```python
from build123d import *

# Parameters (mm, degrees)
BASE_BLOCK_SKETCH_W    = 40
BASE_BLOCK_SKETCH_H    = 20
BASE_BLOCK_DEPTH       = 14
UPRIGHT_SKETCH_W       = 30
UPRIGHT_SKETCH_H       = 20
UPRIGHT_BLOCK_DEPTH    = 51
ANGLED_CUT_30DEG_DEPTH = 51
UPPER_LUG_SKETCH_R     = 3
UPPER_LUG_DEPTH        = 5
LOWER_LUG_SKETCH_R     = 3.5
LOWER_LUG_DEPTH        = 5


with BuildPart() as part:
    # Base Block Sketch → Base Block (new body)
    with BuildSketch(Plane(origin=(0, 0, 0), x_dir=(1, 0, 0), z_dir=(0, 1, 0))):
        with Locations((20, -10)):
            Rectangle(BASE_BLOCK_SKETCH_W, BASE_BLOCK_SKETCH_H)
    extrude(amount=BASE_BLOCK_DEPTH)

    # Upright Sketch → Upright Block (add)
    with BuildSketch(Plane(origin=(0, 14, 0), x_dir=(1, 0, 0), z_dir=(0, 1, 0))):
        with Locations((25, -10)):
            Rectangle(UPRIGHT_SKETCH_W, UPRIGHT_SKETCH_H)
    extrude(amount=UPRIGHT_BLOCK_DEPTH)

    # Angled Cut Sketch 30deg → Angled Cut 30deg (cut)
    with BuildSketch(Plane.XY.offset(20)):
        Polygon((10, 65), (10, 35), (27.320508076, 65), align=None)
    extrude(amount=-ANGLED_CUT_30DEG_DEPTH, mode=Mode.SUBTRACT)

    # Upper Lug Sketch → Upper Lug (add)
    with BuildSketch(Plane.XY.offset(20)):
        with BuildLine():
            Line((27.320508076, 65), (27.320508076, 29.29250995))
            Line((27.320508076, 29.29250995), (75.278835908, 51.655845491))
            ThreePointArc((75.278835908, 51.655845491), (79.154580126, 59.515077298), (72.320508076, 65))
            Line((72.320508076, 65), (27.320508076, 65))
        make_face()
        with Locations((72.320508076, 58)):
            Circle(UPPER_LUG_SKETCH_R, mode=Mode.SUBTRACT)
    extrude(amount=UPPER_LUG_DEPTH)

    # Lower Lug Sketch → Lower Lug (add)
    with BuildSketch(Plane(origin=(0, 0, 0), x_dir=(-1, 0, 0), z_dir=(0, 0, -1))):
        with BuildLine():
            Line((-10, 14), (-55, 14))
            ThreePointArc((-55, 14), (-62, 7), (-55, 0))
            Line((-55, 0), (-10, 0))
            Line((-10, 0), (-10, 14))
        make_face()
        with Locations((-55, 7)):
            Circle(LOWER_LUG_SKETCH_R, mode=Mode.SUBTRACT)
    extrude(amount=LOWER_LUG_DEPTH)


solid = part.part
```
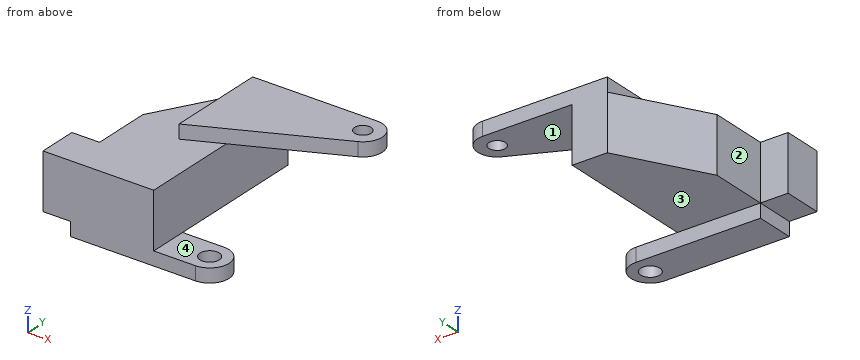
Check sheet for the modelled part. Datum: model origin and axes. Units: mm. Face numbers are marked on the shaded views. A direction names the side the tool comes from. Coordinates: 2 decimals unless noted, no trailing zeros. Write each loop counter-clockwise with the first axis right and the second up, starting at its lowest first coordinate (ties: lowest second). Pieces come first, ordered by that corner, then holes. Notation, with made-up numbers: (-18.5, 68) -> (5.5, 68) arc R29 cw to (5.5, 107) -> close; hole circle Ø10 at (59.5, 69.5). An arc over 180 degrees is marked (long way). Use a Markdown table: item, result.
1. Tool access check on the marked faces 1, 2, 3 and 4. Record the directions out of +Z, -Z, +X, -X, +Y, -Y that give a thin tool (end or side, any length) a straight path to the whole face; none if there is none.
Reported:
| item | result |
|---|---|
| face 1 | -Z, +X, +Y, -Y |
| face 2 | +Z, -Z, -X, +Y |
| face 3 | -Z, +X, -X, +Y |
| face 4 | +Z, +X, +Y, -Y |
2. Go/stop test with flat-tipped pins: pin 1 Ø1 at (y, z) = (44.5, 13) entering from +X; pin 2 Ø4 at (x, z) = (42.5, -1.5) entering from +Y; pin 3 Ø12 at (x, y) = (30, 23.5) entering from +Z; pin 4 Ø9 at (x, y) = (55, 7) entering from -Z. Record where each tip stops, or that it passes through.
Reported:
| item | result |
|---|---|
| pin 1 | stops at x = 40 |
| pin 2 | stops at y = 14 |
| pin 3 | stops at z = 20 |
| pin 4 | stops at z = -5 |
3. Sectioned sample at A-A (y = 7). Enter the section's corners in (x, z), plus the area to 4 significant figures.
Reported:
| item | result |
|---|---|
| outline | (0, 0) -> (10, 0) -> (10, -5) -> (51.5, -5) -> (51.5, 0) -> (40, 0) -> (40, 20) -> (0, 20) -> close; (58.5, -5) -> (62, -5) -> (62, 0) -> (58.5, 0) -> close |
| area | 1,025 mm2 |
4. Sectioned sample at B-B (z = -2). Enter the section's corners in (x, y), plus the area to 3 significant figures.
Reported:
| item | result |
|---|---|
| outline | (10, 0) -> (55, 0) arc R7 ccw to (55, 14) -> (10, 14) -> close; hole circle Ø7 at (55, 7) |
| area | 668 mm2 |
5. Scan lines: line 1 along Y through (x, z) = (55, -2.1); line 2 along Z through (x, y) = (65, 47); line 3 along X through (y, z) = (30.5, 2.75). Record each from-to range of solid material in increasing order.
Reported:
| item | result |
|---|---|
| line 1 | y = 0 to 3.5, 10.5 to 14 |
| line 2 | z = 20 to 25 |
| line 3 | x = 10 to 40 |
6. Sectioned sample at D-D (y = 54). Enter the section's corners in (x, z), plus the area to 3 significant figures.
Reported:
| item | result |
|---|---|
| outline | (20.97, 0) -> (40, 0) -> (40, 20) -> (78.07, 20) -> (78.07, 25) -> (27.32, 25) -> (27.32, 20) -> (20.97, 20) -> close |
| area | 634 mm2 |
7. Sectioned sample at C-C (z = 11.75). Enter the section's corners in (x, y).
Reported:
| item | result |
|---|---|
| outline | (0, 0) -> (40, 0) -> (40, 65) -> (27.32, 65) -> (10, 35) -> (10, 14) -> (0, 14) -> close |
